from build123d import *

# Parameters (mm, degrees)
SKETCH1_R           = 7.5
BOSS_EXTRUDE1_DEPTH = 2.5
SKETCH2_W           = 50
SKETCH2_H           = 20
BOSS_EXTRUDE2_DEPTH = 5


with BuildPart() as part:
    # Sketch1 → Boss-Extrude1 (new, symmetric)
    with BuildSketch(Plane.XY):
        with BuildLine():
            Line((25, 0), (-25, 0))
            Line((-25, 0), (-13.76612817, 25.957660212))
            ThreePointArc((-13.76612817, 25.957660212), (0, 35), (13.76612817, 25.957660212))
            Line((13.76612817, 25.957660212), (25, 0))
        make_face()
        with Locations((0, 20)):
            Circle(SKETCH1_R, mode=Mode.SUBTRACT)
    extrude(amount=BOSS_EXTRUDE1_DEPTH, both=True)

    # Sketch2 → Boss-Extrude2 (add)
    with BuildSketch(Plane.XY.offset(2.5)):
        with Locations((0, -10)):
            Rectangle(SKETCH2_W, SKETCH2_H)
    extrude(amount=-BOSS_EXTRUDE2_DEPTH)


solid = part.part
Build history of the part. All positions in model axes, mm. Give positions to 0.01 mm unless a question says otherwise; leave off trailing zeros. Order: outer loops, then holes, each group sorted by start corner. A loop starts at its lowest first (then second) coordinate and runs counter-clockwise, first axis right, second up. Notation, with made-up numbers: M 3.25,-29 L 56.25,-29 A33 cw 56.25,9 Z; hole C -30,9 d7. An arc over 180 degrees is marked long. Use one line per item in the form item = value.
1) Saw through at A-A (z = -1.6). Give the cut face in (x, y).
Calculated:
outline = M -25,-20 L 25,-20 L 25,0 L 13.77,25.96 A15 ccw -13.77,25.96 L -25,0 Z; hole C 0,20 d15
2) Probe probe 1 along Y at (x, z) = (0, 1.25); probe 2 along Y at (x, z) = (2.5, 1.65); probe 3 along Y at (x, z) = (13.5, 1.65). List the from-to ranges inside material, lowest first.
Calculated:
probe_1 = -20 to 12.5, 27.5 to 35
probe_2 = -20 to 12.93, 27.07 to 34.79
probe_3 = -20 to 26.54
3) Saw through at C-C (y = 20). Give the cut face in (x, z), plus the area to 3 significant figures.
Calculated:
outline = M -16.34,-2.5 L -7.5,-2.5 L -7.5,2.5 L -16.34,2.5 Z; M 7.5,-2.5 L 16.34,-2.5 L 16.34,2.5 L 7.5,2.5 Z
area = 88.4 mm2
4) Drop flat-ended pins along their axis: pin 1 (9 mm diameter, centred on x = 0, y = 20, fed in from -Z); pin 2 (1.5 mm diameter, centred on x = 10, z = -0.5, fed in from +Y). Give the stop position or say it passes through.
Calculated:
pin_1 = through
pin_2 = 31.81
5) Two-plate mould, pull along X, no slides. Class faces 1 (the face through (-0.976, 27.436, -0.035)), 2 (the face through (0, 2, -2.5)), 3 (the face through (-19.46, 12.8, 0.04)): released by +X, released by -X, zero draft, split by the parting line, or undercut.
Calculated:
face_1 = undercut
face_2 = zero draft
face_3 = released by -X
6) Saw through at B-B (x = 0). Give the cut face in (y, z), plus the area to 3 significant figures.
Calculated:
outline = M -20,-2.5 L 12.5,-2.5 L 12.5,2.5 L -20,2.5 Z; M 27.5,-2.5 L 35,-2.5 L 35,2.5 L 27.5,2.5 Z
area = 200 mm2
7) Saw through at D-D (x = 20). Give the cut face in (y, z), plus the area to 3 significant figures.
Calculated:
outline = M -20,-2.5 L 11.55,-2.5 L 11.55,2.5 L -20,2.5 Z
area = 158 mm2
